Check sheet for the modelled part. Datum: model origin and axes. Units: mm. A direction names the side the tool comes from. Round coordinates to 2 decimals unless told otherwise and drop trailing zeros. Order: outer loops, then holes, each group sorted by start corner. A loop starts at its lowest first (then second) coordinate and runs counter-clockwise, first axis right, second up. Notation, with made-up numbers: (0.25, -12.75) -> (51.25, -12.75) arc R33 cw to (51.25, 25.25) -> close; hole circle Ø4 at (50.25, 68). An arc over 180 degrees is marked (long way). Answer in a Markdown table with one row per item. Add a question column.
1. Sectioned sample at A-A, the plane y = 58. Record the boundary of the cut face in (x, z).
2. Sectioned sample at B-B, the plane x = 89. Record the boundary of the cut face in (y, z), then the cut area to 3 significant figures.
3. Sectioned sample at C-C, the plane z = -29.5. Record the boundary of the cut face in (x, y), then the cut area to 3 significant figures.
4. Access from +Z, -Z, +X, -X, +Y, -Y to the whole of each face (thin tool, end or side, straight path). Record for faces 1 (the flat face through (-3, 16, -48)), 2 (the flat face through (120, 239, 8)), 3 (the flat face through (3, 150, -106)).
5. Sectioned sample at D-D, the plane x = -204. Record the boundary of the cut face in (y, z), then the cut area to 3 significant figures.
6. Material ranges on L1, parallel to Z at x = 78, y = 102; L2, parallel to Y at x = -145.5, z = -13.5, recorded low to high. Write a range as from..to.
7. Depth check by flat-ended pin: P1, Ø10, axis at y = 228.5, z = -1, coming from the -X side; P2, Ø13, axis at x = 16.5, z = -106, coming from the +Y side; P3, Ø2, axis at x = 78.5, z = -12, coming from the +Y side. Enter the tip coordinate at first touch or a pass-through.
```python
from build123d import *

# Parameters (mm, degrees)
BOSS_EXTRUDE1_DEPTH = 16
SKETCH2_W           = 500
SKETCH2_H           = 16
BOSS_EXTRUDE2_DEPTH = 130
SKETCH3_W           = 500
SKETCH3_H           = 16
BOSS_EXTRUDE3_DEPTH = 150


with BuildPart() as part:
    # Sketch1 → Boss-Extrude1 (new body)
    with BuildSketch(Plane.XY):
        Polygon((120, 280), (-120, 280), (-120, 200), (-250, 135.697802275), (-250, 0), (250, 0), (250, 135.697802275), (120, 200), align=None)
    extrude(amount=BOSS_EXTRUDE1_DEPTH)

    # Sketch2 → Boss-Extrude2 (add)
    with BuildSketch(Plane.XY.offset(16)):
        with Locations((0, 8)):
            Rectangle(SKETCH2_W, SKETCH2_H)
    extrude(amount=-BOSS_EXTRUDE2_DEPTH)

    # Sketch3 → Boss-Extrude3 (add)
    with BuildSketch(Plane(origin=(0, 0, 0), x_dir=(-1, 0, 0), z_dir=(0, -1, 0))):
        with Locations((0, 106)):
            Rectangle(SKETCH3_W, SKETCH3_H)
    extrude(amount=-BOSS_EXTRUDE3_DEPTH)


solid = part.part
```
Answer key:
| question | item | result |
|---|---|---|
| 1 | outline | (-250, -114) -> (250, -114) -> (250, -98) -> (-250, -98) -> close; (-250, 0) -> (250, 0) -> (250, 16) -> (-250, 16) -> close |
| 2 | outline | (0, -114) -> (150, -114) -> (150, -98) -> (16, -98) -> (16, 0) -> (280, 0) -> (280, 16) -> (0, 16) -> close |
| 2 | area | 8,450 mm² |
| 3 | outline | (-250, 0) -> (250, 0) -> (250, 16) -> (-250, 16) -> close |
| 3 | area | 8,000 mm² |
| 4 | face 1 | +X, -X, +Y |
| 4 | face 2 | +Z, -Z, +X, +Y |
| 4 | face 3 | -Z, +X, -X, +Y |
| 5 | outline | (0, -114) -> (150, -114) -> (150, -98) -> (16, -98) -> (16, 0) -> (158.45, 0) -> (158.45, 16) -> (0, 16) -> close |
| 5 | area | 6,500 mm² |
| 6 | L1 | z = -114..-98, 0..16 |
| 6 | L2 | y = 0..16 |
| 7 | P1 | stops at x = -120 |
| 7 | P2 | stops at y = 150 |
| 7 | P3 | stops at y = 16 |
